Can you work these out from the drawing? Everything is in mm from the part's minimum corner. A direction names the side the tool comes from. Round coordinates to 2 decimals unless told otherwise and drop trailing zeros. Write each loop counter-clockwise with the first axis right and the second up, starting at its lowest first coordinate (ties: lowest second). Pieces come first, ordered by that corner, then holes. Notation, with made-up numbers: (45.5, 42.5) -> (93.5, 42.5) arc R18 cw to (93.5, 74.5) -> close; hole circle Ø5 at (-10, -16). An arc over 180 degrees is marked (long way). Write item = value, one per line. Start each with the question number.
1) Imagine slicing it at D-D, the plane y = 27. Please give me the cut outline in (x, z), then the cut area to 3 significant figures.
2) Imagine slicing it at A-A, the plane y = 67.5. Please give me the cut outline in (x, z).
3) I'm going to push flat-ended pins straight in: pin 1 (2.5 mm diameter, centred on x = 49.5, z = 9, fed in from -Y); pin 2 (5 mm diameter, centred on x = 33, y = 66.5, fed in from -Z); pin 3 (4 mm diameter, centred on x = 10, y = 7.5, fed in from +Z). Where does each tip first touch, or does it pass through?
4) If I drill on line 1 (Y direction, x = 10, z = 3.75); line 2 (Y direction, x = 31, z = 4.25); line 3 (Z direction, x = 33, y = 40.5), over which ranges is the centre line in solid material (lowest first)?
5) For the marked faces 1, 2 and 3, which set-ups out of +Z, -Z, +X, -X, +Y, -Y let a thin tool reach every point of the face, with its end or its side?
6) Imagine slicing it at C-C, the plane x = 54. Please give me the cut outline in (y, z), then the cut area to 3 significant figures.
7) Imagine slicing it at B-B, the plane x = 35. Please give me the cut outline in (y, z).
8) Thinking about a two-plate mould opening in X: for the marked faces 4, 5, 6 and 7, which applies, +X half, -X half, draft (parallel to the pull), parting line (faces both ways), or undercut?
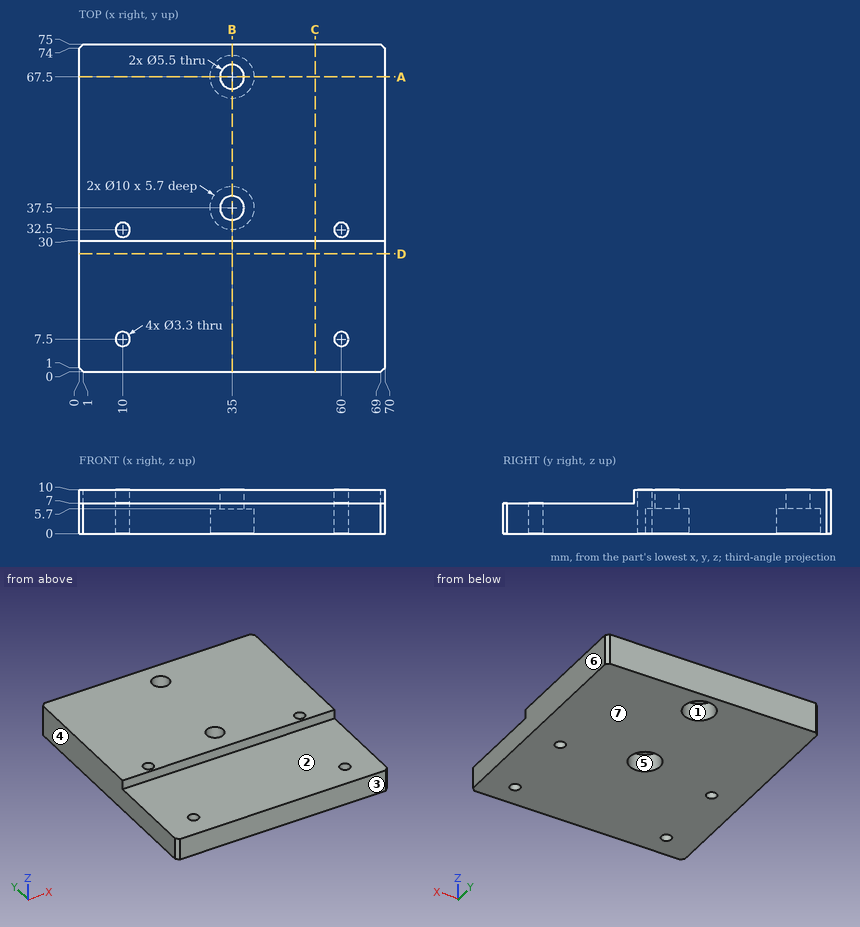
Reported:
q1.outline = (0, 0) -> (70, 0) -> (70, 7) -> (0, 7) -> close
q1.area = 490 mm²
q2.outline = (0, 0) -> (30, 0) -> (30, 5.7) -> (32.25, 5.7) -> (32.25, 10) -> (0, 10) -> close; (37.75, 5.7) -> (40, 5.7) -> (40, 0) -> (70, 0) -> (70, 10) -> (37.75, 10) -> close
q3.pin_1 = 30
q3.pin_2 = 5.7
q3.pin_3 = 7
q4.line_1 = 0 to 5.85, 9.15 to 30.85, 34.15 to 75
q4.line_2 = 0 to 34.5, 40.5 to 64.5, 70.5 to 75
q4.line_3 = 5.7 to 10
q5.face_1 = -Z
q5.face_2 = +Z, +X, -X, -Y
q5.face_3 = +Z, -Z, +X, -X, -Y
q6.outline = (0, 0) -> (75, 0) -> (75, 10) -> (30, 10) -> (30, 7) -> (0, 7) -> close
q6.area = 660 mm²
q7.outline = (0, 0) -> (32.5, 0) -> (32.5, 5.7) -> (34.75, 5.7) -> (34.75, 10) -> (30, 10) -> (30, 7) -> (0, 7) -> close; (40.25, 5.7) -> (42.5, 5.7) -> (42.5, 0) -> (62.5, 0) -> (62.5, 5.7) -> (64.75, 5.7) -> (64.75, 10) -> (40.25, 10) -> close; (70.25, 5.7) -> (72.5, 5.7) -> (72.5, 0) -> (75, 0) -> (75, 10) -> (70.25, 10) -> close
q8.face_4 = -X half
q8.face_5 = undercut
q8.face_6 = +X half
q8.face_7 = draft
